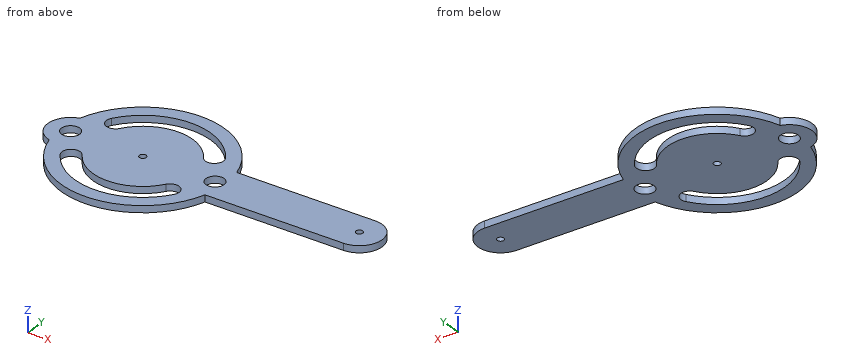
```python
from build123d import *

# Parameters (mm, degrees)
SKETCH_1_R           = 0.75
SKETCH_1_R_2         = 2
BOSS_EXTRUDE_1_DEPTH = 1.5


with BuildPart() as part:
    # Sketch 1 → Boss-Extrude 1 (new body)
    with BuildSketch(Plane.XY):
        with BuildLine():
            Line((48, -5), (17.291616466, -5))
            ThreePointArc((17.291616466, -5), (-0.095597557, -17.99974614), (-17.34375, -4.816049827))
            ThreePointArc((-17.34375, -4.816049827), (-21, 0), (-17.34375, 4.816049827))
            ThreePointArc((-17.34375, 4.816049827), (-0.095597557, 17.99974614), (17.291616466, 5))
            Line((17.291616466, 5), (48, 5))
            ThreePointArc((48, 5), (53, 0), (48, -5))
        make_face()
        Circle(SKETCH_1_R, mode=Mode.SUBTRACT)
        with Locations((16, 0)):
            Circle(SKETCH_1_R_2, mode=Mode.SUBTRACT)
        with Locations((-16, 0)):
            Circle(SKETCH_1_R_2, mode=Mode.SUBTRACT)
        with Locations((48, 0)):
            Circle(SKETCH_1_R, mode=Mode.SUBTRACT)
        with BuildLine():
            ThreePointArc((9.269044534, 5.923243489), (0, 11), (-9.269044534, 5.923243489))
            ThreePointArc((-9.269044534, 5.923243489), (-12.03127872, 5.314916026), (-12.639606182, 8.077150212))
            ThreePointArc((-12.639606182, 8.077150212), (0, 15), (12.639606182, 8.077150212))
            ThreePointArc((12.639606182, 8.077150212), (12.03127872, 5.314916026), (9.269044534, 5.923243489))
        make_face(mode=Mode.SUBTRACT)
        with BuildLine():
            ThreePointArc((-9.269044534, -5.923243489), (-12.03127872, -5.314916026), (-12.639606182, -8.077150212))
            ThreePointArc((-12.639606182, -8.077150212), (0, -15), (12.639606182, -8.077150212))
            ThreePointArc((12.639606182, -8.077150212), (12.03127872, -5.314916026), (9.269044534, -5.923243489))
            ThreePointArc((9.269044534, -5.923243489), (0, -11), (-9.269044534, -5.923243489))
        make_face(mode=Mode.SUBTRACT)
    extrude(amount=BOSS_EXTRUDE_1_DEPTH)


solid = part.part
```
Work out the finished part from the listing and answer in its coordinate system (mm). Give positions to 0.01 mm unless a question says otherwise; leave off trailing zeros. Loops run counter-clockwise (first coordinate to the right, second up) from the corner with the lowest first, then second, coordinate; pieces in that order, holes last. Notation, with made-up numbers: M 72,-32.5 L 123,-32.5 A11 ccw 123,-15.5 Z; hole C 2.25,38 d10. An arc over 180 degrees is marked long. One line per item, written item: value. Start each with the question number.
1. Find section B-B (y = 0). Give the vertices of the cut face in (x, z), and give its area (3 significant figures).
2. This flat-tipped pin is pushed along its axis until it touches: P1, Ø0.8, axis at x = 36, z = 0.5, coming from the +Y side. Where does it stop, or does it pass through?
3. Find the intervals of material crossed by probe 1 along Y at (x, z) = (0, 0.9); probe 2 along Y at (x, z) = (5, 0.45); probe 3 along Y at (x, z) = (10, 1.3), in increasing order.
4. Find section D-D (y = 12.5). Give the vertices of the cut face in (x, z), and give its area (3 significant figures).
5. Find section C-C (z = 0.55). Give the vertices of the cut face in (x, y), and give its area (3 significant figures).
6. Find section A-A (x = 0). Give the vertices of the cut face in (y, z), and give its area (4 significant figures).
Reported:
1. outline: M -21,0 L -18,0 L -18,1.5 L -21,1.5 Z; M -14,0 L -0.75,0 L -0.75,1.5 L -14,1.5 Z; M 0.75,0 L 14,0 L 14,1.5 L 0.75,1.5 Z; M 18,0 L 47.25,0 L 47.25,1.5 L 18,1.5 Z; M 48.75,0 L 53,0 L 53,1.5 L 48.75,1.5 Z
1. area: 94.5 mm²
2. P1: stops at y = 5
3. probe 1: y = -18 to -15, -11 to -0.75, 0.75 to 11, 15 to 18
3. probe 2: y = -17.29 to -14.14, -9.8 to 9.8, 14.14 to 17.29
3. probe 3: y = -14.97 to -11.18, -5.24 to 5.24, 11.18 to 14.97
4. outline: M -12.95,0 L -8.29,0 L -8.29,1.5 L -12.95,1.5 Z; M 8.29,0 L 12.95,0 L 12.95,1.5 L 8.29,1.5 Z
4. area: 14.0 mm²
5. outline: M -17.34,-4.82 A18 ccw 17.29,-5 L 48,-5 A5 ccw 48,5 L 17.29,5 A18 ccw -17.34,4.82 A5 ccw Z; hole C -16,0 d4; hole M -12.64,-8.08 A15 ccw 12.64,-8.08 A2 ccw 9.27,-5.92 A11 cw -9.27,-5.92 A2 ccw Z; hole M -12.64,8.08 A2 ccw -9.27,5.92 A11 cw 9.27,5.92 A2 ccw 12.64,8.08 A15 ccw Z; hole C 0,0 d1.5; hole C 16,0 d4; hole C 48,0 d1.5
5. area: 1,120 mm²
6. outline: M -18,0 L -15,0 L -15,1.5 L -18,1.5 Z; M -11,0 L -0.75,0 L -0.75,1.5 L -11,1.5 Z; M 0.75,0 L 11,0 L 11,1.5 L 0.75,1.5 Z; M 15,0 L 18,0 L 18,1.5 L 15,1.5 Z
6. area: 39.75 mm²
